```python
from build123d import *

# Parameters (mm, degrees)
SKETCH1_W              = 30
SKETCH1_H              = 25
BOSS_EXTRUDE1_DEPTH    = 50
CUT_EXTRUDE1_DEPTH     = 95
M10X1_0_TAPPED_HOLE1_D = 9


with BuildPart() as part:
    # Sketch1 → Boss-Extrude1 (new body)
    with BuildSketch(Plane.XY):
        with Locations((15, 12.5)):
            Rectangle(SKETCH1_W, SKETCH1_H)
    extrude(amount=BOSS_EXTRUDE1_DEPTH)

    # Sketch2 → Cut-Extrude1 (cut)
    with BuildSketch(Plane(origin=(30, 30, 0), x_dir=(0, -1, 0), z_dir=(-1, 0, 0))):
        with BuildLine():
            Line((30, 27), (30, 5))
            ThreePointArc((30, 5), (25.198039027, 16), (30, 27))
        make_face()
    extrude(amount=CUT_EXTRUDE1_DEPTH, mode=Mode.SUBTRACT)

    # M10x1.0 Tapped Hole1 (through all)
    with Locations(Plane(origin=(0, 25, 0), x_dir=(-1, 0, 0), z_dir=(0, 1, 0))):
        with Locations((-15, 37)):
            Hole(M10X1_0_TAPPED_HOLE1_D / 2)


solid = part.part
```
For this review, take the finished solid that the model builds, in its own axes (mm). Give positions to 0.01 mm unless a question says otherwise; leave off trailing zeros. Loops run counter-clockwise (first coordinate to the right, second up) from the corner with the lowest first, then second, coordinate; pieces in that order, holes last. Notation, with made-up numbers: M 67,78.5 L 101,78.5 A18 cw 101,101.5 Z; hole C 52.25,21 d7. An arc over 180 degrees is marked long. One line per item, written item: value. Start each with the question number.
Q1. Draft analysis for pull direction X (two halves, no side actions). For faces 1 (the face through (30, 12, 25)), 2 (the face through (14.02, 12.33, 32.61)), 3 (the face through (11, 0, 41)), state which applies: released by +X, released by -X, zero draft, split by the parting line, or undercut.
Q2. Clearance check with flat-ended pins moving along their axes: pin 1 Ø12 at (y, z) = (16.5, 33) entering from -X; pin 2 Ø3 at (x, z) = (11, 16) entering from -Y; pin 3 Ø8 at (x, z) = (15, 37) entering from -Y. State where each tip first meets the part, or that it passes through.
Q3. Add section B-B (x = 12.25). Give the boundary of the cut face in (y, z).
Q4. Add section C-C (y = 12.75). Give the boundary of the cut face in (x, z), and give its area (3 significant figures).
Q5. For L1, parallel to Z at x = 15, y = 7; L2, parallel to Y at x = 20.75, z = 16; L3, parallel to Z at x = 17.5, y = 19, list the stretches that pass through material, from the lowest coordinate up.
Q6. Add section A-A (z = 37). Give the boundary of the cut face in (x, y), and give its area (3 significant figures).
Q7. Add section D-D (x = 3.5). Give the boundary of the cut face in (y, z).
Reply:
1. face 1: released by +X
1. face 2: undercut
1. face 3: zero draft
2. pin 1: x = 0
2. pin 2: y = 4.73
2. pin 3: through
3. outline: M 0,0 L 25,0 L 25,33.44 L 0,33.44 L 0,27 A15 cw 0,5 Z; M 0,40.56 L 25,40.56 L 25,50 L 0,50 Z
4. outline: M 0,0 L 30,0 L 30,50 L 0,50 Z; hole C 15,37 d9
4. area: 1,440 mm²
5. L1: 0 to 32.5, 41.5 to 50
5. L2: 4.8 to 25
5. L3: 0 to 33.26, 40.74 to 50
6. outline: M 0,0 L 10.5,0 L 10.5,25 L 0,25 Z; M 19.5,0 L 30,0 L 30,25 L 19.5,25 Z
6. area: 525 mm²
7. outline: M 0,0 L 25,0 L 25,50 L 0,50 L 0,27 A15 cw 0,5 Z
